```python
from build123d import *

# Parameters (mm, degrees)
SKETCH1_W           = 986
SKETCH1_H           = 60
BOSS_EXTRUDE1_DEPTH = 30
SKETCH2_W           = 24
SKETCH2_H           = 54
CUT_EXTRUDE1_DEPTH  = 2043


with BuildPart() as part:
    # Sketch1 → Boss-Extrude1 (new body)
    with BuildSketch(Plane.XY):
        Rectangle(SKETCH1_W, SKETCH1_H)
    extrude(amount=BOSS_EXTRUDE1_DEPTH)

    # Sketch2 → Cut-Extrude1 (cut)
    with BuildSketch(Plane.ZY.offset(493)):
        with Locations((15, 0)):
            Rectangle(SKETCH2_W, SKETCH2_H)
    extrude(amount=-CUT_EXTRUDE1_DEPTH, mode=Mode.SUBTRACT)


solid = part.part
```
The model under review builds one solid part; all positions refer to its coordinate system, in mm. A direction names the side the tool comes from. Round coordinates to 2 decimals unless told otherwise and drop trailing zeros. Loops run counter-clockwise (first coordinate to the right, second up) from the corner with the lowest first, then second, coordinate; pieces in that order, holes last.
Item 1: Mouldability with a two-part tool opening along Y and no side actions: class faces 3 (the face through (-7, -30, 15)), 4 (the face through (-7, 0, 30)), 5 (the face through (-7, 0, 3)) as released by +Y, released by -Y, zero draft, split by the parting line, or undercut.
Determined:
face 3: released by -Y
face 4: zero draft
face 5: undercut
Item 2: For line 1 (Z direction, x = -440, y = -16); line 2 (Y direction, x = 68, z = 7.25), list the stretches that pass through material, from the lowest coordinate up.
Determined:
line 1: z = 0 to 3, 27 to 30
line 2: y = -30 to -27, 27 to 30
Item 3: Take a section at A-A (y = -1). Write out the cut boundary in (x, z).
Determined:
outline: (-493, 0) - (493, 0) - (493, 3) - (-493, 3) - close; (-493, 27) - (493, 27) - (493, 30) - (-493, 30) - close
Item 4: Take a section at C-C (x = -122.5). Write out the cut boundary in (y, z), then the cut area to 3 significant figures.
Determined:
outline: (-30, 0) - (30, 0) - (30, 30) - (-30, 30) - close; hole (-27, 3) - (27, 3) - (27, 27) - (-27, 27) - close
area: 504 mm2
Item 5: Take a section at B-B (z = 18.75). Write out the cut boundary in (x, y), then the cut area to 3 significant figures.
Determined:
outline: (-493, -30) - (493, -30) - (493, -27) - (-493, -27) - close; (-493, 27) - (493, 27) - (493, 30) - (-493, 30) - close
area: 5,920 mm2
Item 6: For faces 1 (the face through (-7, 30, 15)), 2 (the face through (-7, 27, 15)), list the 3-axis set-ups (+Z, -Z, +X, -X, +Y, -Y) from which the entire face can be reached by the end or side of a thin tool; tool diameter is ignored.
Determined:
face 1: +Z, -Z, +X, -X, +Y
face 2: +X, -X
